Read the model definition and answer for the solid it produces. Units are mm, in the model's axes. Face numbers are marked on the shaded views. A direction names the side the tool comes from. Round coordinates to 2 decimals unless told otherwise and drop trailing zeros. Write each loop counter-clockwise with the first axis right and the second up, starting at its lowest first coordinate (ties: lowest second). Pieces come first, ordered by that corner, then holes. Notation, with made-up numbers: M -17,43.25 L 14,43.25 A10 ccw 14,56.25 Z; hole C -34.75,48.5 d1. An arc over 180 degrees is marked long. Use one line per item in the form item = value. Start each with the question number.
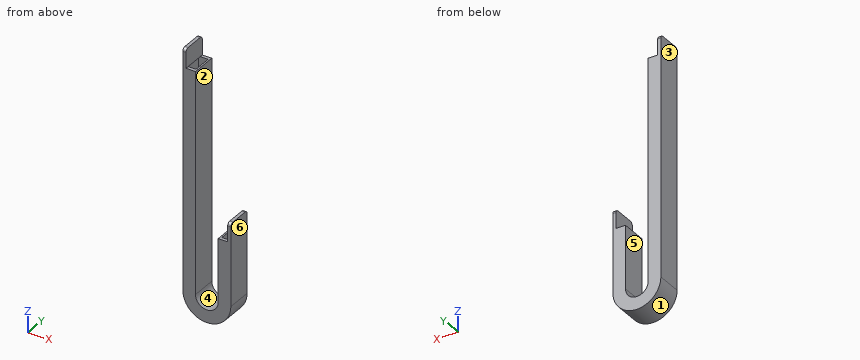
```python
from build123d import *

# Parameters (mm, degrees)
SKETCH_1_W      = 20
SKETCH_1_H      = 40
SKETCH_11_W     = 15
SKETCH_11_H     = 30
SKETCH_3_W      = 5
SKETCH_3_H      = 40
EXTRUDE_1_DEPTH = 30
FILLET_1_R      = 5
SKETCH_5_W      = 5
SKETCH_5_H      = 40
EXTRUDE_2_DEPTH = 30
FILLET_2_R      = 5


with BuildPart() as part:
    # Sweep 1: sweep along a path in 草图2
    with BuildLine(Plane(origin=(0, 0, 0), x_dir=(1, 0, 0), z_dir=(0, 1, 0))) as sweep_1_path:
        Line((0, 0), (0, 350))
        ThreePointArc((0, 350), (28, 378), (56, 350))
        Line((56, 350), (56, 250))
    # 草图1 → Sweep 1 (sweep)
    with BuildSketch(Plane.XY):
        Rectangle(SKETCH_1_W, SKETCH_1_H)
    sweep(path=sweep_1_path.line)

    # Sweep 1 2: sweep along a path in 草图12
    with BuildLine(Plane(origin=(0, 0, 0), x_dir=(1, 0, 0), z_dir=(0, 1, 0))) as sweep_1_2_path:
        Line((0, 0), (0, 350))
        ThreePointArc((0, 350), (28, 378), (56, 350))
        Line((56, 350), (56, 243.98141307))
    # 草图11 → Sweep 1 2 (sweep, cut)
    with BuildSketch(Plane.XY):
        Rectangle(SKETCH_11_W, SKETCH_11_H)
    sweep(path=sweep_1_2_path.line, mode=Mode.SUBTRACT)

    # 草图3 → 凸台-拉伸1 (add)
    with BuildSketch(Plane.XY):
        with Locations((-7.5, 0)):
            Rectangle(SKETCH_3_W, SKETCH_3_H)
    extrude(amount=EXTRUDE_1_DEPTH)

    # 圆角1
    fillet_1_edges = [part.edges().sort_by_distance(p)[0] for p in [
        (-7.5, 20, 30),
        (-7.5, -20, 30),
    ]]
    fillet(fillet_1_edges, radius=FILLET_1_R)

    # 草图5 → 凸台-拉伸2 (add)
    with BuildSketch(Plane.XY.offset(-250)):
        with Locations((63.5, 0)):
            Rectangle(SKETCH_5_W, SKETCH_5_H)
    extrude(amount=EXTRUDE_2_DEPTH)

    # 圆角2
    fillet_2_edges = [part.edges().sort_by_distance(p)[0] for p in [
        (63.5, 20, -220),
        (63.5, -20, -220),
    ]]
    fillet(fillet_2_edges, radius=FILLET_2_R)


solid = part.part
```
Q1. Find section C-C on x = 28. Write down the section's boundary in (y, z).
Q2. Straight lines are drawn through the part: line 1 (X direction, y = 9.5, z = -266.5); line 2 (X direction, y = 10, z = -239); line 3 (Y direction, x = 60.5, z = -347). For each, find the intervals that lie inside material, in ascending order. Write a range as [from, to].
Q3. For a pull along X with two mould halves and no side action, classify the marked faces 1, 2, 3 and 4 as +X half, -X half, draft (parallel to the pull), parting line (faces both ways), or undercut.
Q4. Find section B-B on y = -11.5. Write down the section's boundary in (x, z), and give its area (3 significant figures).
Q5. Find section A-A on z = -240. Write down the section's boundary in (x, y), and give its area (3 significant figures).
Q6. Each of these flat-tipped pins is pushed along its axis until it touches: pin 1 Ø6 at (y, z) = (-12.5, -108) entering from +X; pin 2 Ø10 at (x, y) = (20.5, -14) entering from -Z; pin 3 Ø6 at (x, y) = (36.5, 8.5) entering from +Z. Where does it stop, or does it pass through?
Q7. Find section D-D on z = -120. Write down the section's boundary in (x, y).
Q8. A tool of negligible diameter and unlimited length cuts with its end or side. For the marked faces 5 and 6, from which of +Z, -Z, +X, -X, +Y, -Y can it reach the whole face along a straight path? Write none if from no direction.
Response:
q1.outline = M -20,-388 L 20,-388 L 20,-368 L -20,-368 Z; hole M -15,-385.5 L 15,-385.5 L 15,-370.5 L -15,-370.5 Z
q2.line_1 = [-10, -7.5], [7.5, 10], [46, 48.5], [63.5, 66]
q2.line_2 = [-10, -7.5], [7.5, 10], [61, 66]
q2.line_3 = [-20, -15], [15, 20]
q3.face_1 = parting line
q3.face_2 = undercut
q3.face_3 = -X half
q3.face_4 = undercut
q4.outline = M -10,-350 A38 ccw 66,-350 L 66,-220 L 61,-220 L 61,-250 L 63.5,-250 L 63.5,-350 A35.5 cw -7.5,-350 L -7.5,0 L -5,0 L -5,30 L -10,30 Z; M 7.5,-350 A20.5 ccw 48.5,-350 L 48.5,-250 L 46,-250 L 46,-350 A18 cw 10,-350 L 10,0 L 7.5,0 Z
q4.area = 2,990 mm²
q5.outline = M -10,-20 L 10,-20 L 10,20 L -10,20 Z; M 61,-20 L 66,-20 L 66,20 L 61,20 Z; hole M -7.5,-15 L 7.5,-15 L 7.5,15 L -7.5,15 Z
q5.area = 550 mm²
q6.pin_1 = 10
q6.pin_2 = -387.92
q6.pin_3 = -363.85
q7.outline = M -10,-20 L 10,-20 L 10,20 L -10,20 Z; hole M -7.5,-15 L 7.5,-15 L 7.5,15 L -7.5,15 Z
q8.face_5 = +Z, +Y, -Y
q8.face_6 = +Z, -Z, +X, +Y, -Y
